```python
from build123d import *

# Parameters (mm, degrees)
SKETCH1_W           = 28
SKETCH1_H           = 28
SKETCH1_W_2         = 0.581812165
SKETCH1_H_2         = 3.033734858
BOSS_EXTRUDE1_DEPTH = 27
SKETCH2_W           = 28
SKETCH2_H           = 28
BOSS_EXTRUDE2_DEPTH = 2
SKETCH3_R           = 3
CUT_EXTRUDE1_DEPTH  = 6
SKETCH4_R           = 1.5
CUT_EXTRUDE2_DEPTH  = 25
FILLET1_R           = 1
SKETCH5_R           = 10
SKETCH5_R_2         = 5
EXTRUDE_THIN1_DEPTH = 15
BOSS_EXTRUDE3_DEPTH = 4
CUT_EXTRUDE3_START  = -1
SKETCH7_R           = 10
SKETCH7_R_2         = 7
CUT_EXTRUDE3_DEPTH  = 1
SKETCH8_R           = 6
CUT_EXTRUDE4_DEPTH  = 22
SKETCH9_W           = 8.469861182
SKETCH9_H           = 8.944508274
CUT_EXTRUDE5_DEPTH  = 15


with BuildPart() as part:
    # Sketch1 → Boss-Extrude1 (new body)
    with BuildSketch(Plane.XY):
        with Locations((17, 0)):
            Rectangle(SKETCH1_W, SKETCH1_H)
        Polygon((18.5, 7.071580399), (18.5, 6.29199588), (18.76385967, 6.29199588), (18.76385967, 6.681788139), (21.23614033, 6.681788139), (21.23614033, 6.29199588), (21.5, 6.29199588), (21.5, 7.071580399), align=None, mode=Mode.SUBTRACT)
        with Locations((10.815679405, 0)):
            Rectangle(SKETCH1_W_2, SKETCH1_H_2, mode=Mode.SUBTRACT)
        Polygon((18.5, -6.29199588), (18.5, -7.071580399), (21.5, -7.071580399), (21.5, -6.29199588), (21.23614033, -6.29199588), (21.23614033, -6.681788139), (18.76385967, -6.681788139), (18.76385967, -6.29199588), align=None, mode=Mode.SUBTRACT)
    extrude(amount=BOSS_EXTRUDE1_DEPTH)

    # Sketch2 → Boss-Extrude2 (add)
    with BuildSketch(Plane.XY.offset(27)):
        with Locations((17, 0)):
            Rectangle(SKETCH2_W, SKETCH2_H)
    extrude(amount=-BOSS_EXTRUDE2_DEPTH)

    # Sketch3 → Cut-Extrude1 (cut)
    with BuildSketch(Plane.XY.offset(27)):
        with Locations((17, 0)):
            Circle(SKETCH3_R)
    extrude(amount=-CUT_EXTRUDE1_DEPTH, mode=Mode.SUBTRACT)

    # Sketch4 → Cut-Extrude2 (cut)
    with BuildSketch(Plane.XY.offset(21)):
        with Locations((17, 0)):
            Circle(SKETCH4_R)
    extrude(amount=-CUT_EXTRUDE2_DEPTH, mode=Mode.SUBTRACT)

    # Fillet1
    fillet1_edges = [part.edges().sort_by_distance(p)[0] for p in [
        (3, 0, 27),
        (17, -14, 27),
        (31, 0, 27),
        (17, -14, 0),
        (3, 0, 0),
        (17, 14, 0),
        (31, 0, 0),
        (31, -14, 13.5),
        (3, -14, 13.5),
        (3, 14, 13.5),
        (31, 14, 13.5),
        (17, 14, 27),
    ]]
    fillet(fillet1_edges, radius=FILLET1_R)

    # Sketch5 → Extrude-Thin1 (add)
    with BuildSketch(Plane(origin=(31, 0, 0), x_dir=(0, 0, -1), z_dir=(1, 0, 0))):
        with Locations((-13.5, 0)):
            Circle(SKETCH5_R)
        with Locations((-13.5, 0)):
            Circle(SKETCH5_R_2, mode=Mode.SUBTRACT)
    extrude(amount=EXTRUDE_THIN1_DEPTH)

    # Sketch6 → Boss-Extrude3 (add)
    with BuildSketch(Plane(origin=(46, 0, 0), x_dir=(0, 0, -1), z_dir=(1, 0, 0))):
        Polygon((-23.296433781, 0), (-18.398216891, -8.483960521), (-8.601783109, -8.483960521), (-3.703566219, 0), (-8.601783109, 8.483960521), (-18.398216891, 8.483960521), align=None)
    extrude(amount=BOSS_EXTRUDE3_DEPTH)

    # Sketch7 → Cut-Extrude3 (cut)
    with BuildSketch(Plane(origin=(46, 0, 0), x_dir=(0, 0, -1), z_dir=(1, 0, 0)).offset(CUT_EXTRUDE3_START)):
        with Locations(Location((-13.5, 0, 0), (0, 0, 270))):
            Circle(SKETCH7_R)
        with Locations(Location((-13.5, 0, 0), (0, 0, 90))):
            Circle(SKETCH7_R_2, mode=Mode.SUBTRACT)
    extrude(amount=CUT_EXTRUDE3_DEPTH, mode=Mode.SUBTRACT)

    # Sketch8 → Cut-Extrude4 (cut)
    with BuildSketch(Plane(origin=(50, 0, 0), x_dir=(0, 0, -1), z_dir=(1, 0, 0))):
        with Locations((-13.5, 0)):
            Circle(SKETCH8_R)
    extrude(amount=-CUT_EXTRUDE4_DEPTH, mode=Mode.SUBTRACT)

    # Sketch9 → Cut-Extrude5 (cut)
    with BuildSketch(Plane(origin=(0, 0, 0), x_dir=(-1, 0, 0), z_dir=(0, 0, -1))):
        with Locations((-17, 0)):
            Rectangle(SKETCH9_W, SKETCH9_H)
    extrude(amount=-CUT_EXTRUDE5_DEPTH, mode=Mode.SUBTRACT)


solid = part.part
```
For this review, take the finished solid that the model builds, in its own axes (mm). A direction names the side the tool comes from. Round coordinates to 2 decimals unless told otherwise and drop trailing zeros. Write each loop counter-clockwise with the first axis right and the second up, starting at its lowest first coordinate (ties: lowest second). Pieces come first, ordered by that corner, then holes. Notation, with made-up numbers: M -38.5,-8 L 16.5,-8 A15 ccw 16.5,2 Z; hole C 13,69 d3. An arc over 180 degrees is marked long. One line per item, written item: value. Start each with the question number.
(1) Machinability: for faces 4 (the flat face through (20, 6.682, 12)), 5 (the flat face through (47.972, 4.183, 6.118)), 6 (the flat face through (48, -8.484, 14)), 7 (the flat face through (18.3, -1.3, 21)), which of the approach directions +Z, -Z, +X, -X, +Y, -Y give a long, thin tool a straight path to every point of the face, cutting with its end or side? Answer none if there is none.
(2) Wall thickness on line 1 (X direction, y = -0.75, z = 11.25); line 2 (X direction, y = -7.75, z = 17.25); line 3 (X direction, y = -2, z = 8.75): over which ranges is each line inside the solid? List them lowest first.
(3) We need section A-A (x = 17). Give the boundary of the cut face in (y, z), and give its area (3 significant figures).
(4) We need section C-C (x = 31.5). Give the boundary of the cut face in (y, z), and give its area (3 significant figures).
(5) Insertion check: pin 1 (5 mm diameter, centred on x = 17, y = 0, fed in from -Z); pin 2 (12 mm diameter, centred on x = 40, y = 1, fed in from +Z); pin 3 (1 mm diameter, centred on y = -3, z = 13, fed in from +X). Each pin has a flat end and moves straight along its axis. Give the tip position at first contact, or say it passes through.
(6) We need section B-B (z = 13.5). Count the separate pieces of the cut face and the enclosed holes in it, and give its area (3 significant figures).
(7) The part is to be moulded in two halves that separate along Y. For faces 1 (the cylindrical face through (17.182, 13.715, 0.301)), 2 (the flat face through (17, -4.472, 7)), 3 (the flat face through (17, -14, 13)), say which applies: released by +Y, released by -Y, zero draft, split by the parting line, or undercut.
(8) We need section D-D (y = 9). Give the boundary of the cut face in (x, z).
Result:
1. face 4: -Z
1. face 5: -Z, +X, +Y
1. face 6: +Z, -Z, +X, -Y
1. face 7: +Z
2. line 1: 3 to 10.52, 11.11 to 12.77, 21.23 to 28
2. line 2: 3 to 45, 46 to 50
2. line 3: 3 to 12.77, 21.23 to 28
3. outline: M -14,1 A1 ccw -13,0 L -4.47,0 L -4.47,15 L -1.5,15 L -1.5,21 L -3,21 L -3,27 L -13,27 A1 ccw -14,26 Z; M 1.5,15 L 4.47,15 L 4.47,0 L 13,0 A1 ccw 14,1 L 14,26 A1 ccw 13,27 L 3,27 L 3,21 L 1.5,21 Z
3. area: 567 mm²
4. outline: C 0,13.5 d20; hole C 0,13.5 d12
4. area: 201 mm²
5. pin 1: z = 15
5. pin 2: z = 23.5
5. pin 3: x = 28
6. separate pieces: 1
6. enclosed holes: 4
6. area: 801 mm²
7. face 1: released by +Y
7. face 2: undercut
7. face 3: released by -Y
8. outline: M 3,1 A1 ccw 4,0 L 30,0 A1 ccw 31,1 L 31,9.14 L 45,9.14 L 45,17.86 L 31,17.86 L 31,26 A1 ccw 30,27 L 4,27 A1 ccw 3,26 Z
